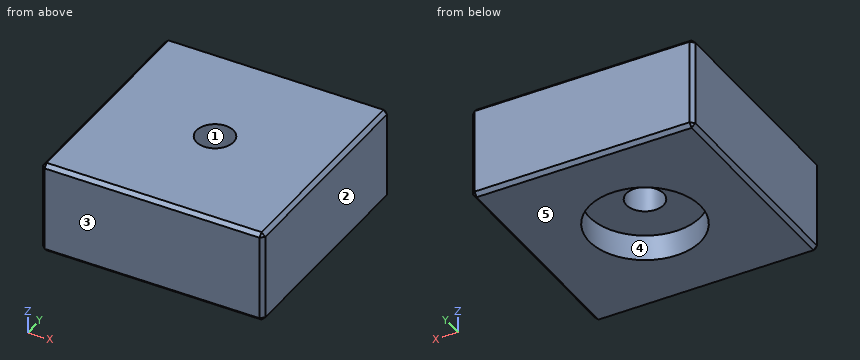
from build123d import *

# Parameters (mm, degrees)
SKETCH1_W           = 60
SKETCH1_H           = 60
BOSS_EXTRUDE1_DEPTH = 25
CHAMFER1_SIZE       = 1
SKETCH2_R           = 15
CUT_EXTRUDE1_DEPTH  = 7
SKETCH3_R           = 5
CUT_EXTRUDE2_DEPTH  = 47.086874487


with BuildPart() as part:
    # Sketch1 → Boss-Extrude1 (new body)
    with BuildSketch(Plane.XY):
        Rectangle(SKETCH1_W, SKETCH1_H)
    extrude(amount=BOSS_EXTRUDE1_DEPTH)

    # Chamfer1
    chamfer1_edges = [part.edges().sort_by_distance(p)[0] for p in [
        (30, 0, 25),
        (0, -30, 25),
        (-30, 0, 25),
        (0, -30, 0),
        (30, 0, 0),
        (0, 30, 0),
        (-30, 0, 0),
        (0, 30, 25),
        (-30, -30, 12.5),
        (30, -30, 12.5),
        (30, 30, 12.5),
        (-30, 30, 12.5),
    ]]
    chamfer(chamfer1_edges, length=CHAMFER1_SIZE)

    # Sketch2 → Cut-Extrude1 (cut)
    with BuildSketch(Plane(origin=(0, 0, 0), x_dir=(-1, 0, 0), z_dir=(0, 0, -1))):
        Circle(SKETCH2_R)
    extrude(amount=-CUT_EXTRUDE1_DEPTH, mode=Mode.SUBTRACT)

    # Sketch3 → Cut-Extrude2 (cut, through all)
    with BuildSketch(Plane(origin=(0, 0, 7), x_dir=(-1, 0, 0), z_dir=(0, 0, -1))):
        Circle(SKETCH3_R)
    extrude(amount=-CUT_EXTRUDE2_DEPTH, mode=Mode.SUBTRACT)


solid = part.part
Could you check a few things on this model? Use its own coordinates, in mm. Face numbers are marked on the shaded views. A direction names the side the tool comes from. Coordinates: 2 decimals unless noted, no trailing zeros. Write each loop counter-clockwise with the first axis right and the second up, starting at its lowest first coordinate (ties: lowest second). Pieces come first, ordered by that corner, then holes. Notation, with made-up numbers: (-29.5, 60) - (11.5, 60) arc R29 cw to (11.5, 82) - close; hole circle Ø10 at (36.25, 49). An arc over 180 degrees is marked (long way). Put each result on its own line as item: value. Start each with the question number.
Q1. Which directions (+Z, -Z, +X, -X, +Y, -Y) give clear straight access to the entire face, cutting with the end or side of a thin tool? Please do the marked faces 4 and 5.
Q2. Thinking about a two-plate mould opening in X: for the marked faces 1, 2 and 3, which applies, pulls with the +X half, pulls with the -X half, needs draft (parallel to the pull), parting line crosses it, or undercut?
Q3. Please list where these lines run through material, in increasing order: L1, parallel to Y at x = 0, z = 15.5; L2, parallel to Y at x = 0, z = 4; L3, parallel to Z at x = -6.5, y = -11.
Q4. I want a section at B-B on z = 17. Write out the boundary of the cut face in (x, y), plus the area to 3 significant figures.
Q5. I'm going to push a flat-ended pin straight in: P1, Ø13, axis at x = 0, y = 0, coming from the -Z side. Where does the tip first touch, or does it pass through?
Q6. I want a section at A-A on y = 0. Write out the boundary of the cut face in (x, z).
Q7. I want a section at D-D on y = 7.5. Write out the boundary of the cut face in (x, z).
Checks:
1. face 4: -Z
1. face 5: -Z, +X, -X, +Y, -Y
2. face 1: undercut
2. face 2: pulls with the +X half
2. face 3: needs draft
3. L1: -30 to -5, 5 to 30
3. L2: -30 to -15, 15 to 30
3. L3: 7 to 25
4. outline: (-30, -29) - (-29, -30) - (29, -30) - (30, -29) - (30, 29) - (29, 30) - (-29, 30) - (-30, 29) - close; hole circle Ø10 at (0, 0)
4. area: 3,520 mm²
5. P1: z = 7
6. outline: (-30, 1) - (-29, 0) - (-15, 0) - (-15, 7) - (-5, 7) - (-5, 25) - (-29, 25) - (-30, 24) - close; (5, 7) - (15, 7) - (15, 0) - (29, 0) - (30, 1) - (30, 24) - (29, 25) - (5, 25) - close
7. outline: (-30, 1) - (-29, 0) - (-12.99, 0) - (-12.99, 7) - (12.99, 7) - (12.99, 0) - (29, 0) - (30, 1) - (30, 24) - (29, 25) - (-29, 25) - (-30, 24) - close
